Design review of the part shown in the three views and the two pictorial views. Dimensions are in mm from the part's minimum x, y and z. Round coordinates to 2 decimals unless told otherwise and drop trailing zeros. Loops run counter-clockwise (first coordinate to the right, second up) from the corner with the lowest first, then second, coordinate; pieces in that order, holes last. Notation, with made-up numbers: M 44.5,34.5 L 100.5,34.5 A18 cw 100.5,63.5 Z; hole C -31,-12 d1. An arc over 180 degrees is marked long. Return JSON: item names as keys, results as strings. Group by question number.
Q1. Clearance check with a flat-ended pin moving along its axis: pin 1 Ø1.5 at (x, z) = (1.5, 12) entering from +Y. State where the tip first meets the part, or that it passes through.
Q2. Consider section A-A (z = 30). State the section outline as (x, y) points.
Q3. To check wall thickness, follow line 1 along Y through (x, z) = (3, 6); line 2 along Z through (x, y) = (5.5, 3.1); line 3 along X through (y, z) = (4.1, 6). State the ranges of each line that lie inside material, in increasing order.
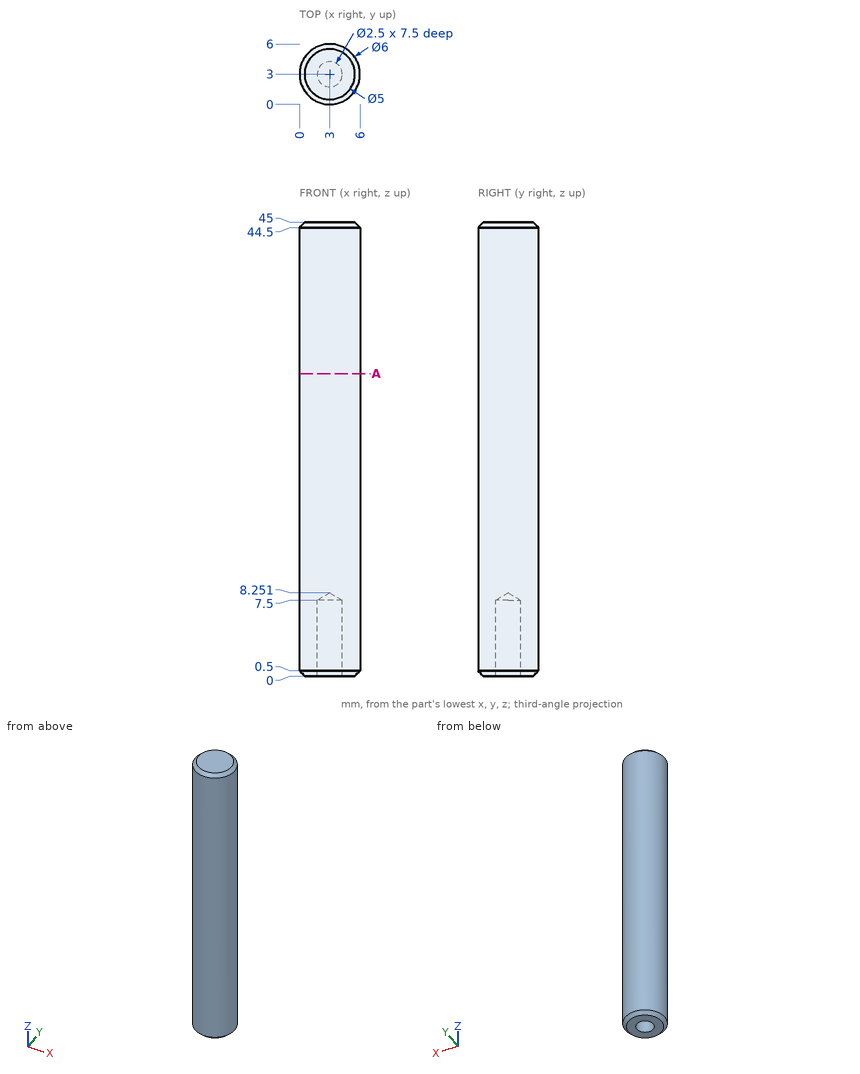
Values:
{
 "1": {"pin 1": "stops at y = 5.9"},
 "2": {"outline": "C 3,3 d6"},
 "3": {"line 1": "y = 0 to 1.75, 4.25 to 6", "line 2": "z = 0 to 45", "line 3": "x = 0.21 to 2.41, 3.59 to 5.79"}
}
